Part print with two shaded views. Sizes in mm from the minimum x, y, z corner. A direction names the side the tool comes from. Round coordinates to 2 decimals unless told otherwise and drop trailing zeros. Loops run counter-clockwise (first coordinate to the right, second up) from the corner with the lowest first, then second, coordinate; pieces in that order, holes last. Notation, with made-up numbers: M 24.25,21 L 66.25,21 A11 ccw 66.25,41 Z; hole C 79,-0.5 d3. An arc over 180 degrees is marked long. Use a Markdown table: item, result. Add a question column.
Item 1: Pin check, flat tips, straight feed: P1, Ø4, axis at y = 10.5, z = 122.5, coming from the +X side; P2, Ø8, axis at x = 115, z = 15, coming from the +Y side. Stop position of each tip, or through.
Item 2: Saw through at C-C on y = 14.5. Write the cut outline in (x, z).
Item 3: Saw through at B-B on x = 15. Write the cut outline in (y, z).
Item 4: Saw through at D-D on z = 39. Write the cut outline in (x, y), then the cut area to 3 significant figures.
Item 5: Wall check: L1, parallel to X at y = 4.5, z = 140; L2, parallel to X at y = 13.75, z = 76.5; L3, parallel to X at y = 10.75, z = 18.5. Give the ranges that are in metal, low to high. Write a range as from..to.
Item 6: Tool access for the marked faces 1 and 2: list every direction of +Z, -Z, +X, -X, +Y, -Y with a clear straight run to the whole face (end or side of a thin tool).
Item 7: Saw through at A-A on z = 15. Write the cut outline in (x, y).
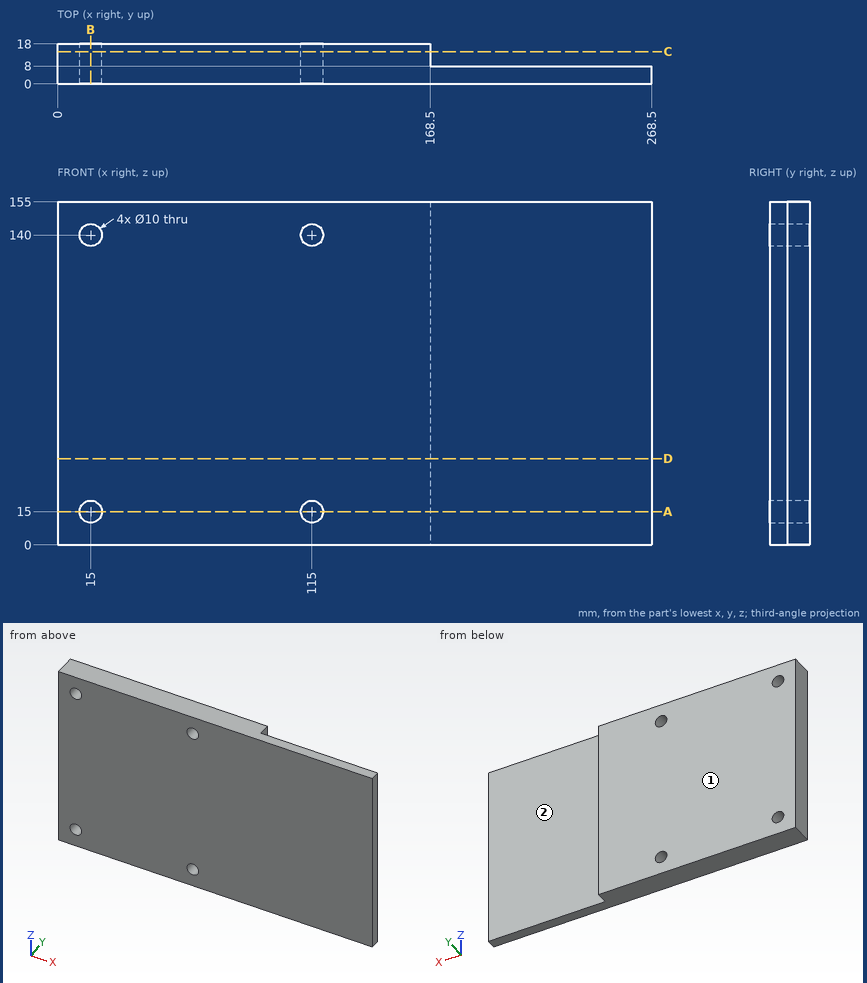
Entries:
| question | item | result |
|---|---|---|
| 1 | P1 | x = 168.5 |
| 1 | P2 | through |
| 2 | outline | M 0,0 L 168.5,0 L 168.5,155 L 0,155 Z; hole C 15,15 d10; hole C 15,140 d10; hole C 115,15 d10; hole C 115,140 d10 |
| 3 | outline | M 0,0 L 18,0 L 18,10 L 0,10 Z; M 0,20 L 18,20 L 18,135 L 0,135 Z; M 0,145 L 18,145 L 18,155 L 0,155 Z |
| 4 | outline | M 0,0 L 268.5,0 L 268.5,8 L 168.5,8 L 168.5,18 L 0,18 Z |
| 4 | area | 3,830 mm2 |
| 5 | L1 | 0..10, 20..110, 120..268.5 |
| 5 | L2 | 0..168.5 |
| 5 | L3 | 0..11.43, 18.57..111.43, 118.57..168.5 |
| 6 | face 1 | +Z, -Z, +X, -X, +Y |
| 6 | face 2 | +Z, -Z, +X, +Y |
| 7 | outline | M 0,0 L 10,0 L 10,18 L 0,18 Z; M 20,0 L 110,0 L 110,18 L 20,18 Z; M 120,0 L 268.5,0 L 268.5,8 L 168.5,8 L 168.5,18 L 120,18 Z |
